CAD build for the part. Positions are in the model's coordinates, mm. A direction names the side the tool comes from. Give positions to 0.01 mm unless a question says otherwise; leave off trailing zeros. Write each loop counter-clockwise with the first axis right and the second up, starting at its lowest first coordinate (ties: lowest second). Pieces come first, ordered by that corner, then holes. Notation, with made-up numbers: (82.25, 50) - (103.25, 50) arc R23 ccw to (103.25, 62) - close; hole circle Ø5 at (55.25, 18). An arc over 180 degrees is marked (long way). Write item = value, one per line. Start each with the question number.
```python
from build123d import *

# Parameters (mm, degrees)
SKETCH_1_W                = 120
SKETCH_1_H                = 200
EXTRUDE_1_DEPTH           = 10
CHAMFER_1_SIZE            = 3
HOLE_WIZARD_0_D           = 5.5
HOLE_WIZARD_0_DEPTH       = 10.1
HOLE_WIZARD_0_CBORE_D     = 10
HOLE_WIZARD_0_CBORE_DEPTH = 5.7
HOLE_WIZARD_0_TIP         = 1.652366702
SKETCH_4_W                = 38
SKETCH_4_H                = 90
SKETCH_4_W_2              = 8
CUT_EXTRUDE_1_DEPTH       = 20
CHAMFER_2_SIZE            = 2
FILLET_1_R                = 3
HOLE_WIZARD_M4_1_D        = 3.3
HOLE_WIZARD_M4_1_DEPTH    = 10.1
HOLE_WIZARD_M4_1_TIP      = 0.991420021
HOLE_WIZARD_M4_2_D        = 3.3
HOLE_WIZARD_M4_2_DEPTH    = 10.1
HOLE_WIZARD_M4_2_TIP      = 0.991420021
MM_2_D                    = 4
MM_2_DEPTH                = 12.4
MM_2_TIP                  = 1.201721238
HOLE_WIZARD_M5_2_D        = 4.2
HOLE_WIZARD_M5_2_DEPTH    = 12.4
HOLE_WIZARD_M5_2_TIP      = 1.2618073
HOLE_WIZARD_M5_3_D        = 4.2
HOLE_WIZARD_M5_3_DEPTH    = 12.4
HOLE_WIZARD_M5_3_TIP      = 1.2618073


with BuildPart() as part:
    # 草图1 → 凸台-拉伸1 (new body)
    with BuildSketch(Plane(origin=(0, 0, 0), x_dir=(1, 0, 0), z_dir=(0, 1, 0))):
        Rectangle(SKETCH_1_W, SKETCH_1_H)
    extrude(amount=EXTRUDE_1_DEPTH)

    # 倒角1
    chamfer_1_edges = [part.edges().sort_by_distance(p)[0] for p in [
        (60, 5, 100),
        (-60, 5, 100),
        (-60, 5, -100),
        (60, 5, -100),
    ]]
    chamfer(chamfer_1_edges, length=CHAMFER_1_SIZE)

    # 打孔尺寸(%根据)内六角圆柱头螺钉的类型0
    with Locations(Plane(origin=(0, 10, 0), x_dir=(1, 0, 0), z_dir=(0, 1, 0))):
        with Locations((-52, 83), (-52, 53), (22, 53), (22, 83)):
            CounterBoreHole(HOLE_WIZARD_0_D / 2, HOLE_WIZARD_0_CBORE_D / 2, HOLE_WIZARD_0_CBORE_DEPTH, depth=HOLE_WIZARD_0_DEPTH)
            with Locations((0, 0, -(HOLE_WIZARD_0_DEPTH + HOLE_WIZARD_0_TIP / 2))):  # 118° drill point
                Cone(0, HOLE_WIZARD_0_D / 2, HOLE_WIZARD_0_TIP, mode=Mode.SUBTRACT)

    # 草图4 → 切除-拉伸1 (cut)
    with BuildSketch(Plane(origin=(0, 10, 0), x_dir=(1, 0, 0), z_dir=(0, 1, 0))):
        with Locations((41, -55)):
            Rectangle(SKETCH_4_W, SKETCH_4_H)
        with Locations((-56, -55)):
            Rectangle(SKETCH_4_W_2, SKETCH_4_H)
    extrude(amount=-CUT_EXTRUDE_1_DEPTH, mode=Mode.SUBTRACT)

    # 倒角2
    chamfer_2_edges = [part.edges().sort_by_distance(p)[0] for p in [
        (22, 5, 100),
        (60, 5, 10),
        (-60, 5, 10),
        (-52, 5, 100),
    ]]
    chamfer(chamfer_2_edges, length=CHAMFER_2_SIZE)

    # 圆角1
    fillet_1_edges = [part.edges().sort_by_distance(p)[0] for p in [
        (22, 5, 10),
        (-52, 5, 10),
    ]]
    fillet(fillet_1_edges, radius=FILLET_1_R)

    # M4 螺纹孔1
    with Locations(Plane.ZY.offset(52)):
        with Locations((30, 5), (60, 5), (90, 5)):
            Hole(HOLE_WIZARD_M4_1_D / 2, depth=HOLE_WIZARD_M4_1_DEPTH)
            with Locations((0, 0, -(HOLE_WIZARD_M4_1_DEPTH + HOLE_WIZARD_M4_1_TIP / 2))):  # 118° drill point
                Cone(0, HOLE_WIZARD_M4_1_D / 2, HOLE_WIZARD_M4_1_TIP, mode=Mode.SUBTRACT)

    # M4 螺纹孔2
    with Locations(Plane(origin=(22, 0, 0), x_dir=(0, 0, -1), z_dir=(1, 0, 0))):
        with Locations((-30, 5), (-60, 5), (-90, 5)):
            Hole(HOLE_WIZARD_M4_2_D / 2, depth=HOLE_WIZARD_M4_2_DEPTH)
            with Locations((0, 0, -(HOLE_WIZARD_M4_2_DEPTH + HOLE_WIZARD_M4_2_TIP / 2))):  # 118° drill point
                Cone(0, HOLE_WIZARD_M4_2_D / 2, HOLE_WIZARD_M4_2_TIP, mode=Mode.SUBTRACT)

    # 大小mm 暗销孔2
    with Locations(Plane(origin=(0, 10, 0), x_dir=(1, 0, 0), z_dir=(0, 1, 0))):
        with Locations((43, 12), (43, -4)):
            Hole(MM_2_D / 2, depth=MM_2_DEPTH)
            with Locations((0, 0, -(MM_2_DEPTH + MM_2_TIP / 2))):  # 118° drill point
                Cone(0, MM_2_D / 2, MM_2_TIP, mode=Mode.SUBTRACT)

    # M5 螺纹孔2
    with Locations(Plane(origin=(0, 10, 0), x_dir=(1, 0, 0), z_dir=(0, 1, 0))):
        with Locations((53, -4), (33, -4), (53, 12), (33, 12)):
            Hole(HOLE_WIZARD_M5_2_D / 2, depth=HOLE_WIZARD_M5_2_DEPTH)
            with Locations((0, 0, -(HOLE_WIZARD_M5_2_DEPTH + HOLE_WIZARD_M5_2_TIP / 2))):  # 118° drill point
                Cone(0, HOLE_WIZARD_M5_2_D / 2, HOLE_WIZARD_M5_2_TIP, mode=Mode.SUBTRACT)

    # M5 螺纹孔3
    with Locations(Plane(origin=(0, 10, 0), x_dir=(1, 0, 0), z_dir=(0, 1, 0))):
        with Locations((52, 55), (37, 55), (52, 75), (37, 75)):
            Hole(HOLE_WIZARD_M5_3_D / 2, depth=HOLE_WIZARD_M5_3_DEPTH)
            with Locations((0, 0, -(HOLE_WIZARD_M5_3_DEPTH + HOLE_WIZARD_M5_3_TIP / 2))):  # 118° drill point
                Cone(0, HOLE_WIZARD_M5_3_D / 2, HOLE_WIZARD_M5_3_TIP, mode=Mode.SUBTRACT)


solid = part.part
```
1. Cut at C-C (z = 40). Give the cut face in (x, y).
2. Cut at B-B (x = 33). Give the cut face in (y, z).
3. Cut at A-A (z = 4). Give the cut face in (x, y), then the cut area to 3 significant figures.
4. Wall check: line 1 along Z through (x, y) = (37, 6); line 2 along X through (y, z) = (5.65, -83); line 3 along X through (y, z) = (2.9, -83). Give the ranges that are in metal, low to high.
5. Pin check, flat tips, straight feed: pin 1 Ø0.9 at (x, y) = (-57, 3) entering from +Z; pin 2 Ø2 at (y, z) = (5, 60) entering from +X; pin 3 Ø3 at (y, z) = (5, 30) entering from +X; pin 4 Ø2.5 at (x, z) = (43, 4) entering from -Y. Stop position of each tip, or through.
6. Tool access for faces 4 (the cylindrical face through (34.666, 4.93, 5.278)), 5 (the cylindrical face through (20.92, 7.19, -78.12)): list every direction of +Z, -Z, +X, -X, +Y, -Y with a clear straight run to the whole face (end or side of a thin tool).
7. Mould opens along X. For faces 1 (the flat face through (-52, 5, 56)), 2 (the flat face through (22, 5, 56)), 3 (the cylindrical face through (51.06, 4.93, 4.8)) say: +X half, -X half, draft (parallel to the pull), parting line (faces both ways), or undercut.
Output:
q1.outline = (-52, 0) - (22, 0) - (22, 10) - (-52, 10) - close
q2.outline = (0, -100) - (10, -100) - (10, -14.1) - (0, -14.1) - close; (0, -9.9) - (10, -9.9) - (10, 1.9) - (0, 1.9) - close; (0, 6.1) - (10, 6.1) - (10, 10) - (0, 10) - close
q3.outline = (-60, 0) - (30.9, 0) - (30.9, 10) - (-60, 10) - close; (35.1, 0) - (41, 0) - (41, 10) - (35.1, 10) - close; (45, 0) - (50.9, 0) - (50.9, 10) - (45, 10) - close; (55.1, 0) - (60, 0) - (60, 10) - (55.1, 10) - close
q3.area = 1,080 mm2
q4.line_1 = -100 to -77.1, -72.9 to -57.1, -52.9 to 10
q4.line_2 = -60 to -57, -47 to 17, 27 to 60
q4.line_3 = -60 to -54.75, -49.25 to 19.25, 24.75 to 60
q5.pin_1 = 10
q5.pin_2 = 11.51
q5.pin_3 = 11.81
q5.pin_4 = through
q6.face_4 = +Y, -Y
q6.face_5 = +Y
q7.face_1 = -X half
q7.face_2 = +X half
q7.face_3 = undercut
